from build123d import *

# Parameters (mm, degrees)
SKETCH1_R           = 2.3
BOSS_EXTRUDE1_DEPTH = 20
SKETCH3_W           = 0.694541754
SKETCH3_H           = 0.2
BOSS_EXTRUDE2_START = 2
SKETCH4_R           = 2.3
BOSS_EXTRUDE2_DEPTH = 2
SKETCH5_R           = 2.5
BOSS_EXTRUDE3_DEPTH = 10
SKETCH6_W           = 1
SKETCH6_H           = 1.000091558
SKETCH10_R          = 2.5
BOSS_EXTRUDE4_DEPTH = 6
SKETCH11_W          = 1
SKETCH11_H          = 1
BOSS_EXTRUDE5_START = 1
SKETCH12_R          = 2.5
BOSS_EXTRUDE5_DEPTH = 1


with BuildPart() as part:
    # Sketch1 → Boss-Extrude1 (new body)
    with BuildSketch(Plane(origin=(0, 0, 0), x_dir=(0, 0, -1), z_dir=(1, 0, 0))):
        Circle(SKETCH1_R)
    extrude(amount=BOSS_EXTRUDE1_DEPTH)

    # Sketch3 → Revolve1 (revolve)
    with BuildSketch(Plane.XY, mode=Mode.PRIVATE) as revolve1_sk:
        with Locations((10.347270877, 2.4)):
            Rectangle(SKETCH3_W, SKETCH3_H)
    revolve(revolve1_sk.sketch.rotate(Axis((20, 0, 0), (-1, 0, 0)), 270), axis=Axis((20, 0, 0), (-1, 0, 0)))

    # Sketch4 → Boss-Extrude2 (add)
    with BuildSketch(Plane.ZY.offset(BOSS_EXTRUDE2_START)):
        Circle(SKETCH4_R)
    extrude(amount=-BOSS_EXTRUDE2_DEPTH)

    # Sketch5 → Boss-Extrude3 (add)
    with BuildSketch(Plane(origin=(20, 0, 0), x_dir=(0, 0, -1), z_dir=(1, 0, 0))):
        with Locations(Location((0, 0, 0), (0, 0, 180))):
            Circle(SKETCH5_R)
    extrude(amount=-BOSS_EXTRUDE3_DEPTH)

    # Sketch6 → Cut-Revolve1 (revolve, cut)
    with BuildSketch(Plane(origin=(0.993947206, 0, 0), x_dir=(1, 0, 0), z_dir=(0, 0, 1)), mode=Mode.PRIVATE) as cut_revolve1_sk:
        with Locations((17.5, 1.999954221)):
            Rectangle(SKETCH6_W, SKETCH6_H)
    revolve(cut_revolve1_sk.sketch.rotate(Axis((20.993947206, 0, 0), (-1, 0, 0)), 270), axis=Axis((20.993947206, 0, 0), (-1, 0, 0)), mode=Mode.SUBTRACT)

    # Sketch10 → Boss-Extrude4 (add)
    with BuildSketch(Plane.ZY.offset(-10)):
        Circle(SKETCH10_R)
    extrude(amount=BOSS_EXTRUDE4_DEPTH)

    # Sketch11 → Revolve2 (revolve)
    with BuildSketch(Plane.XY, mode=Mode.PRIVATE) as revolve2_sk:
        with Locations((10.5, 3)):
            Rectangle(SKETCH11_W, SKETCH11_H)
    revolve(revolve2_sk.sketch.rotate(Axis((20, 0, 0), (-1, 0, 0)), 90), axis=Axis((20, 0, 0), (-1, 0, 0)))

    # Sketch12 → Boss-Extrude5 (add)
    with BuildSketch(Plane(origin=(20, 0, 0), x_dir=(0, 0, -1), z_dir=(1, 0, 0)).offset(BOSS_EXTRUDE5_START)):
        Circle(SKETCH12_R)
    extrude(amount=-BOSS_EXTRUDE5_DEPTH)


solid = part.part
The model under review builds one solid part; all positions refer to its coordinate system, in mm. A direction names the side the tool comes from. Give positions to 0.01 mm unless a question says otherwise; leave off trailing zeros. Order: outer loops, then holes, each group sorted by start corner. A loop starts at its lowest first (then second) coordinate and runs counter-clockwise, first axis right, second up. Notation, with made-up numbers: M 38.5,59 L 82.5,59 A11 ccw 82.5,76 Z; hole C 74.5,-22.5 d10. An arc over 180 degrees is marked long. Use one line per item in the form item = value. Start each with the question number.
Item 1: We need section B-B on z = -2. Give the boundary of the cut face in (x, y).
Item 2: Insertion check: pin 1 Ø1.5 at (y, z) = (1, 3) entering from -X; pin 2 Ø2 at (x, z) = (10.5, -1.5) entering from +Y. Each pin has a flat end and moves straight along its axis. Give the tip position at first contact, or say it passes through.
Item 3: The part is to be moulded in two halves that separate along X. For faces 4 (the cylindrical face through (7.04, -2.44, -0.54)), 5 (the flat face through (10, 2, 2)), 6 (the flat face through (17.994, -2, 0)), say which applies: pulls with the +X half, pulls with the -X half, needs draft (parallel to the pull), parting line crosses it, or undercut.
Item 4: For faces 1 (the flat face through (18.994, -2, 0)), 2 (the cylindrical face through (10.507, 3.105, -1.615)), 3 (the cylindrical face through (14.5, -0.1, -2.5)), list the 3-axis set-ups (+Z, -Z, +X, -X, +Y, -Y) from which the entire face can be reached by the end or side of a thin tool; tool diameter is ignored.
Item 5: To check wall thickness, follow line 1 along X through (y, z) = (1, -2.25); line 2 along X through (y, z) = (-1, -2); line 3 along X through (y, z) = (-2.75, -2). State the ranges of each line that lie inside material, in increasing order. Write a range as from..to.
Item 6: We need section A-A on y = 0. Give the boundary of the cut face in (x, z).
Completed:
q1.outline = M -2,-1.14 L 4,-1.14 L 4,-1.5 L 10,-1.5 L 10,-2.87 L 11,-2.87 L 11,-1.5 L 17.99,-1.5 L 17.99,1.5 L 11,1.5 L 11,2.87 L 10,2.87 L 10,1.5 L 4,1.5 L 4,1.14 L -2,1.14 Z; M 18.99,-1.5 L 21,-1.5 L 21,1.5 L 18.99,1.5 Z
q2.pin_1 = 4
q2.pin_2 = 3.46
q3.face_4 = needs draft
q3.face_5 = pulls with the -X half
q3.face_6 = undercut
q4.face_1 = none
q4.face_2 = +X, -X
q4.face_3 = +X
q5.line_1 = 4..17.99, 18.99..21
q5.line_2 = -2..17.99, 18.99..21
q5.line_3 = 10..11
q6.outline = M -2,-2.3 L 4,-2.3 L 4,-2.5 L 10,-2.5 L 10,-3.5 L 11,-3.5 L 11,-2.5 L 17.99,-2.5 L 17.99,-1.5 L 18.99,-1.5 L 18.99,-2.5 L 21,-2.5 L 21,2.5 L 18.99,2.5 L 18.99,1.5 L 17.99,1.5 L 17.99,2.5 L 11,2.5 L 11,3.5 L 10,3.5 L 10,2.5 L 4,2.5 L 4,2.3 L -2,2.3 Z
